from build123d import *

# Parameters (mm, degrees)
SKETCH1_W         = 2
SKETCH1_H         = 12.5
CIRPATTERN1_COUNT = 3


with BuildPart() as part:
    # Sketch1 → Revolve1 (revolve)
    with BuildSketch(Plane(origin=(0, 0, 0), x_dir=(0, 0, -1), z_dir=(1, 0, 0)), mode=Mode.PRIVATE) as revolve1_sk:
        with Locations((1, 13.75)):
            Rectangle(SKETCH1_W, SKETCH1_H)
    revolve(revolve1_sk.sketch.rotate(Axis((0, 0, 4.366666667), (0, 0, -1)), 90), axis=Axis((0, 0, 4.366666667), (0, 0, -1)))

    # Sketch2 → Cut-Revolve1 (revolve, cut)
    with BuildSketch(Plane(origin=(0, 0, 0), x_dir=(0, 0, -1), z_dir=(1, 0, 0)), mode=Mode.PRIVATE) as cut_revolve1_sk:
        Polygon((0, 19.25), (2, 17.25), (2, 15), (0, 15), align=None)
    cut_revolve1 = revolve(cut_revolve1_sk.sketch.rotate(Axis((0, 15, 0.909195932), (0, 0, -1)), 90), axis=Axis((0, 15, 0.909195932), (0, 0, -1)), mode=Mode.SUBTRACT)

    # CirPattern1: Cut-Revolve1 ×3 about axis
    cirpattern1_axis = Axis((0, 0, 0), (0, 0, 1))
    for i in range(1, CIRPATTERN1_COUNT):
        add(cut_revolve1.rotate(cirpattern1_axis, i * 360 / CIRPATTERN1_COUNT), mode=Mode.SUBTRACT)


solid = part.part
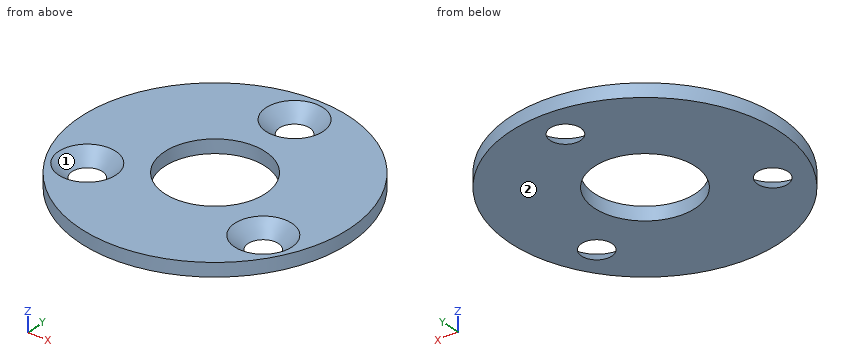
The listing builds one solid part. Answer for the finished solid, in the listing's coordinates (mm). Face numbers are marked on the shaded views. Round coordinates to 2 decimals unless told otherwise and drop trailing zeros. Write each loop counter-clockwise with the first axis right and the second up, starting at its lowest first coordinate (ties: lowest second). Pieces come first, ordered by that corner, then holes. Notation, with made-up numbers: M -8,3.5 L 8,3.5 A14 cw 8,25.5 Z; hole C 55,-39 d3. An arc over 180 degrees is marked long. Write each question's results on one line, items separated by ' | '. Start each with the question number.
Item 1: Find section D-D on y = 15. Write down the section's boundary in (x, z).
Item 2: Straight lines are drawn through the part: probe 1 along X at (y, z) = (-10.5, -0.35); probe 2 along X at (y, z) = (-6, -0.95); probe 3 along Y at (x, z) = (0, -0.75). For each, find the intervals that lie inside material, in ascending order.
Item 3: Find section A-A on y = 0. Write down the section's boundary in (x, z).
Item 4: Given pin 1 Ø1 at (x, z) = (14, -0.5) entering from +Y; pin 2 Ø8 at (x, y) = (-5.5, 2) entering from +Z; pin 3 Ø1.5 at (x, y) = (-16, 14) entering from -Z, each flat-ended and moving along its own axis, determine where each tip first touches the part or whether it passes through.
Item 5: Find section B-B on x = 0. Write down the section's boundary in (y, z), and give its area (3 significant figures).
Item 6: The mould has two halves that part along X. Classify the marked faces 1 and 2: +X half, -X half, draft (parallel to the pull), parting line (faces both ways), or undercut.
Item 7: Find section C-C on z = -0.35. Write down the section's boundary in (x, y), and give its area (3 significant figures).
Answer block:
1) outline: M -13.23,-2 L -2.25,-2 L -4.25,0 L -13.23,0 Z; M 2.25,-2 L 13.23,-2 L 13.23,0 L 4.25,0 Z
2) probe 1: x = -17.02 to -15.48, -10.5 to 10.5, 15.48 to 17.02 | probe 2: x = -19.08 to -15.93, -10.05 to -4.5, 4.5 to 10.05, 15.93 to 19.08 | probe 3: y = -20 to -7.5, 7.5 to 11.5, 18.5 to 20
3) outline: M -20,-2 L -7.5,-2 L -7.5,0 L -20,0 Z; M 7.5,-2 L 20,-2 L 20,0 L 7.5,0 Z
4) pin 1: stops at y = 14.76 | pin 2: stops at z = 0 | pin 3: passes through
5) outline: M -20,-2 L -7.5,-2 L -7.5,0 L -20,0 Z; M 7.5,-2 L 12.75,-2 L 10.75,0 L 7.5,0 Z; M 17.25,-2 L 20,-2 L 20,0 L 19.25,0 Z | area: 37.0 mm²
6) face 1: undercut | face 2: draft
7) outline: C 0,0 d40; hole C -12.99,-7.5 d7.8; hole C 0,0 d15; hole C 0,15 d7.8; hole C 12.99,-7.5 d7.8 | area: 937 mm²
